from build123d import *

# Parameters (mm, degrees)
BASE_PLATE_SKETCH_W              = 100
BASE_PLATE_SKETCH_H              = 100
BASE_PLATE_SKETCH_R              = 22.5
BASE_PLATE_100X100_BORE_45_DEPTH = 10
SIDE_RAILS_SKETCH_W              = 155
SIDE_RAILS_SKETCH_H              = 32
SIDE_RAILS_DEPTH                 = 20
END_BLOCKS_SKETCH_W              = 20
END_BLOCKS_SKETCH_H              = 32
END_BLOCKS_20X20_DEPTH           = 10


with BuildPart() as part:
    # Base Plate Sketch → Base Plate 100x100 Bore Ø45 (new body)
    with BuildSketch(Plane(origin=(0, 0, 0), x_dir=(1, 0, 0), z_dir=(0, 1, 0))):
        Rectangle(BASE_PLATE_SKETCH_W, BASE_PLATE_SKETCH_H)
        with Locations(Location((0, 0, 0), (0, 0, 270))):
            Circle(BASE_PLATE_SKETCH_R, mode=Mode.SUBTRACT)
    extrude(amount=BASE_PLATE_100X100_BORE_45_DEPTH)

    # Side Rails Sketch → Side Rails (add)
    with BuildSketch(Plane.XZ):
        with Locations((19.5, 42)):
            Rectangle(SIDE_RAILS_SKETCH_W, SIDE_RAILS_SKETCH_H)
        with Locations((19.5, -42)):
            Rectangle(SIDE_RAILS_SKETCH_W, SIDE_RAILS_SKETCH_H)
    extrude(amount=SIDE_RAILS_DEPTH)

    # End Blocks Sketch → End Blocks 20x20 (add)
    with BuildSketch(Plane(origin=(0, 0, 0), x_dir=(1, 0, 0), z_dir=(0, 1, 0))):
        with Locations((87, 42)):
            Rectangle(END_BLOCKS_SKETCH_W, END_BLOCKS_SKETCH_H)
        with Locations((87, -42)):
            Rectangle(END_BLOCKS_SKETCH_W, END_BLOCKS_SKETCH_H)
    extrude(amount=END_BLOCKS_20X20_DEPTH)


solid = part.part
The listing builds one solid part. Answer for the finished solid, in the listing's coordinates (mm). A direction names the side the tool comes from. Give positions to 0.01 mm unless a question says otherwise; leave off trailing zeros. Write each loop counter-clockwise with the first axis right and the second up, starting at its lowest first coordinate (ties: lowest second). Pieces come first, ordered by that corner, then holes.
1) Given P1, Ø11, axis at x = -8, y = 4, coming from the -Z side; P2, Ø3, axis at y = 4.5, z = -16, coming from the +X side; P3, Ø12, axis at x = 33.5, z = -12, coming from the -Y side; P4, Ø5, axis at y = 3, z = -45.5, coming from the -X side, each flat-ended and moving along its own axis, determine where each tip first touches the part or whether it passes through.
2) Section D-D (x = 0) is taken. Write down the section's boundary in (y, z), and give its area (3 significant figures).
3) Section C-C (x = 43.5) is taken. Write down the section's boundary in (y, z).
4) Section B-B (z = 0) is taken. Write down the section's boundary in (x, y).
5) A tool of negligible diameter and unlimited length cuts with its end or side. For faces 4 (the face through (77, 5, -42)), 5 (the face through (-1, 5, -50)), 6 (the face through (-23, 0, 0)), 7 (the face through (-50, 5, 1)), from which of +Z, -Z, +X, -X, +Y, -Y can it reach the whole face along a straight path? Write none if from no direction.
6) For a pull along Z with two mould halves and no side action, classify faces 1 (the face through (87, 10, -42)), 2 (the face through (18, -8, 26)), 3 (the face through (18, -8, 58)) as pulls with the +Z half, pulls with the -Z half, needs draft (parallel to the pull), parting line crosses it, or undercut.
7) Section A-A (y = 3.25) is taken. Write down the section's boundary in (x, z).
8) Find the intervals of material crossed by L1, parallel to X at y = 3.5, z = -49.5; L2, parallel to X at y = 5.5, z = 0; L3, parallel to Y at x = -35.5, z = -10, in increasing order.
Response:
1. P1: stops at z = -58
1. P2: stops at x = 50
1. P3: stops at y = 0
1. P4: stops at x = -50
2. outline: (-20, -58) - (0, -58) - (0, -50) - (10, -50) - (10, -22.5) - (0, -22.5) - (0, -26) - (-20, -26) - close; (-20, 26) - (0, 26) - (0, 22.5) - (10, 22.5) - (10, 50) - (0, 50) - (0, 58) - (-20, 58) - close
2. area: 1,830 mm2
3. outline: (-20, -58) - (0, -58) - (0, -50) - (10, -50) - (10, 50) - (0, 50) - (0, 58) - (-20, 58) - (-20, 26) - (0, 26) - (0, -26) - (-20, -26) - close
4. outline: (-50, 0) - (-22.5, 0) - (-22.5, 10) - (-50, 10) - close; (22.5, 0) - (50, 0) - (50, 10) - (22.5, 10) - close
5. face 4: +Z, -Z, +Y
5. face 5: -Z, -X, +Y
5. face 6: +X, -X, -Y
5. face 7: +Z, -Z, -X, +Y
6. face 1: needs draft
6. face 2: undercut
6. face 3: pulls with the +Z half
7. outline: (-50, -50) - (50, -50) - (50, 50) - (-50, 50) - close; (77, -58) - (97, -58) - (97, -26) - (77, -26) - close; (77, 26) - (97, 26) - (97, 58) - (77, 58) - close; hole circle Ø45 at (0, 0)
8. L1: x = -50 to 50, 77 to 97
8. L2: x = -50 to -22.5, 22.5 to 50
8. L3: y = 0 to 10
